Read the model definition and answer for the solid it produces. Units are mm, in the model's axes. Coordinates: 2 decimals unless noted, no trailing zeros. Write each loop counter-clockwise with the first axis right and the second up, starting at its lowest first coordinate (ties: lowest second). Pieces come first, ordered by that corner, then holes. Notation, with made-up numbers: (-35.75, 32.25) -> (14.25, 32.25) arc R23 cw to (14.25, 49.25) -> close; hole circle Ø9 at (-27, 21.25). An arc over 180 degrees is marked (long way). Answer in a Markdown table with one row per item. Add a question column.
Item 1: Section A-A on x = -960 is taken. Write down the section's boundary in (y, z).
Item 2: For a pull along Z with two mould halves and no side action, classify faces 1 (the face through (-472.19, -0.06, -237.2)), 2 (the face through (-16, 4, -9)) as +Z half, -Z half, draft (parallel to the pull), parting line (faces both ways), or undercut.
Item 3: Section B-B on z = -262 is taken. Write down the section's boundary in (x, y).
Item 4: Straight lines are drawn through the part: line 1 (X direction, y = -1, z = -262); line 2 (X direction, y = -0.25, z = 143); line 3 (Z direction, x = -503.5, y = 3). For each, find the intervals that lie inside material, in ascending order. Write a range as from..to.
```python
from build123d import *

# Parameters (mm, degrees)
SKETCH_1_W      = 2324
SKETCH_1_H      = 1330
SKETCH_1_R      = 26
SKETCH_1_R_2    = 10
EXTRUDE_1_DEPTH = 4


with BuildPart() as part:
    # 草图1 → 凸台-拉伸1 (new, symmetric)
    with BuildSketch(Plane(origin=(0, 0, 0), x_dir=(1, 0, 0), z_dir=(0, 1, 0))):
        Rectangle(SKETCH_1_W, SKETCH_1_H)
        with Locations(Location((-480, 262, 0), (0, 0, 270))):
            Circle(SKETCH_1_R, mode=Mode.SUBTRACT)
        with Locations(Location((0, 537, 0), (0, 0, 270))):
            Circle(SKETCH_1_R_2, mode=Mode.SUBTRACT)
        with Locations(Location((0, -143, 0), (0, 0, 270))):
            Circle(SKETCH_1_R_2, mode=Mode.SUBTRACT)
        with Locations(Location((-960, 262, 0), (0, 0, 270))):
            Circle(SKETCH_1_R, mode=Mode.SUBTRACT)
    extrude(amount=EXTRUDE_1_DEPTH, both=True)


solid = part.part
```
Results below:
| question | item | result |
|---|---|---|
| 1 | outline | (-4, -665) -> (4, -665) -> (4, -288) -> (-4, -288) -> close; (-4, -236) -> (4, -236) -> (4, 665) -> (-4, 665) -> close |
| 2 | face 1 | undercut |
| 2 | face 2 | draft |
| 3 | outline | (-1162, -4) -> (-986, -4) -> (-986, 4) -> (-1162, 4) -> close; (-934, -4) -> (-506, -4) -> (-506, 4) -> (-934, 4) -> close; (-454, -4) -> (1162, -4) -> (1162, 4) -> (-454, 4) -> close |
| 4 | line 1 | x = -1162..-986, -934..-506, -454..1162 |
| 4 | line 2 | x = -1162..-10, 10..1162 |
| 4 | line 3 | z = -665..-273.12, -250.88..665 |
